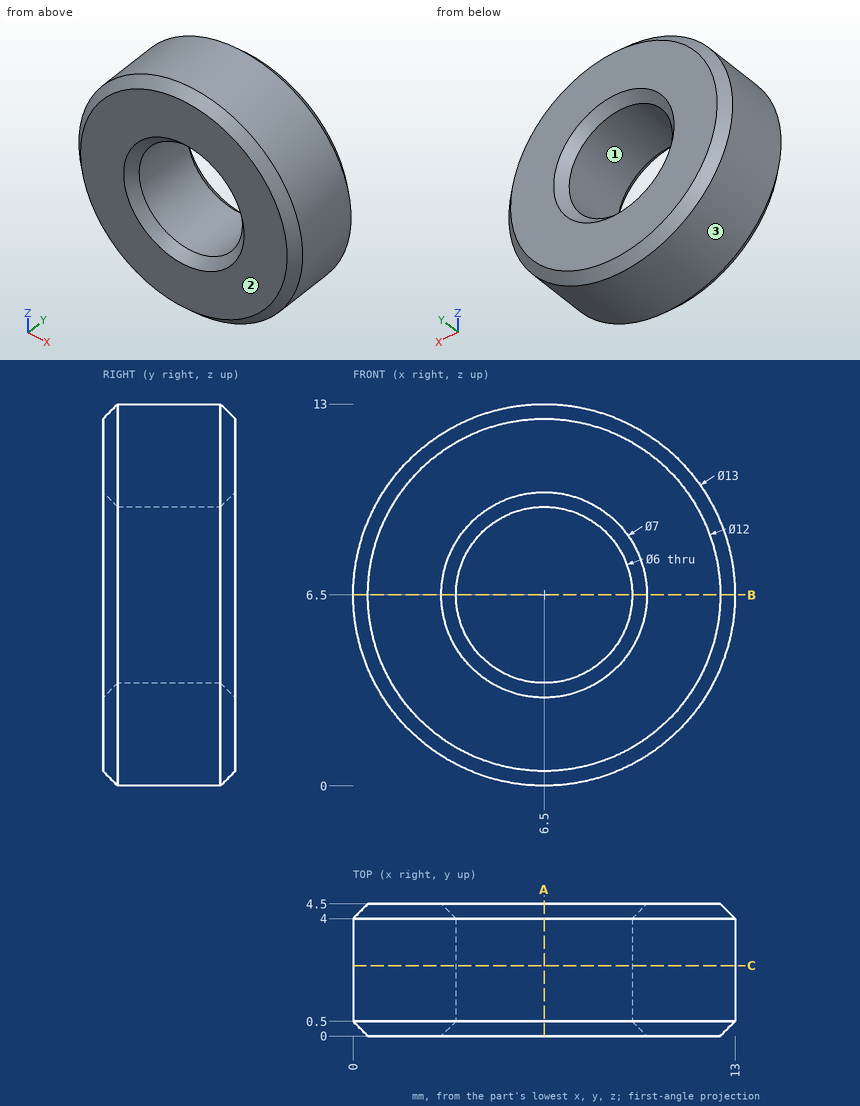
Verification items for this drawing (mm, ordinates from the low corner). Give positions to 0.01 mm unless a question says otherwise; leave off trailing zeros. Write each loop counter-clockwise with the first axis right and the second up, starting at its lowest first coordinate (ties: lowest second). Pieces come first, ordered by that corner, then holes. Notation, with made-up numbers: (80, -33) -> (102, -33) arc R35 ccw to (102, 6) -> close; hole circle Ø5 at (15, -11.75). An arc over 180 degrees is marked (long way). Use CSV: the item, a comma, the result in double quotes. Start each with the question number.
Q1. Cross-section at A-A on x = 6.5. Enter the section's corners in (y, z), and give its area (3 significant figures).
Q2. Release check for a two-part mould opening along Z. For the marked faces 1, 2 and 3 record: +Z half, -Z half, draft (parallel to the pull), parting line (faces both ways), or undercut.
Q3. Cross-section at B-B on z = 6.5. Enter the section's corners in (x, y), and give its area (3 significant figures).
Q4. Depth check by flat-ended pin: P1, Ø1.5, axis at x = 2, y = 2.5, coming from the +Z side; P2, Ø2, axis at x = 3, y = 2, coming from the -Z side; P3, Ø1.5, axis at y = 4, z = 5, coming from the -X side. Enter the tip coordinate at first touch or a pass-through.
Q5. Scan lines: line 1 along X through (y, z) = (1.4, 6.5); line 2 along X through (y, z) = (2.3, 8.5); line 3 along Z through (x, y) = (6.75, 1.6). Record each from-to range of solid material in increasing order.
Q6. Cross-section at C-C on y = 2.4. Enter the section's corners in (x, z), and give its area (3 significant figures).
Working result:
1,outline,"(0, 0.5) -> (0.5, 0) -> (4, 0) -> (4.5, 0.5) -> (4.5, 3) -> (4, 3.5) -> (0.5, 3.5) -> (0, 3) -> close; (0, 10) -> (0.5, 9.5) -> (4, 9.5) -> (4.5, 10) -> (4.5, 12.5) -> (4, 13) -> (0.5, 13) -> (0, 12.5) -> close"
1,area,"30.5 mm^2"
2,face 1,"undercut"
2,face 2,"draft"
2,face 3,"parting line"
3,outline,"(0, 0.5) -> (0.5, 0) -> (3, 0) -> (3.5, 0.5) -> (3.5, 4) -> (3, 4.5) -> (0.5, 4.5) -> (0, 4) -> close; (9.5, 0.5) -> (10, 0) -> (12.5, 0) -> (13, 0.5) -> (13, 4) -> (12.5, 4.5) -> (10, 4.5) -> (9.5, 4) -> close"
3,area,"30.5 mm^2"
4,P1,"stops at z = 11.81"
4,P2,"stops at z = 0.5"
4,P3,"stops at x = 0.04"
5,line 1,"x = 0 to 3.5, 9.5 to 13"
5,line 2,"x = 0.32 to 4.26, 8.74 to 12.68"
5,line 3,"z = 0 to 3.51, 9.49 to 13"
6,outline,"circle Ø13 at (6.5, 6.5); hole circle Ø6 at (6.5, 6.5)"
6,area,"104 mm^2"
